```python
from build123d import *

# Parameters (mm, degrees)
SKETCH1_W                                    = 40
SKETCH1_H                                    = 430
BOSS_EXTRUDE1_DEPTH                          = 7.5
SKETCH2_R                                    = 6.5
CUT_EXTRUDE1_DEPTH                           = 3
HEX_SOCKET_CAP_SCREW_HOLE_TYPE_1_D           = 6.6
HEX_SOCKET_CAP_SCREW_HOLE_TYPE_1_CBORE_D     = 11
HEX_SOCKET_CAP_SCREW_HOLE_TYPE_1_CBORE_DEPTH = 6.8
M5_TAPPED_HOLE1_D                            = 4.2
M5_TAPPED_HOLE1_DEPTH                        = 15
M5_TAPPED_HOLE1_TIP                          = 1.2618073
CHAMFER1_SIZE                                = 2
HEX_SOCKET_CAP_SCREW_HOLE_TYPE_2_D           = 6.6
HEX_SOCKET_CAP_SCREW_HOLE_TYPE_2_CBORE_D     = 11
HEX_SOCKET_CAP_SCREW_HOLE_TYPE_2_CBORE_DEPTH = 6.8
M6_TAPPED_HOLE1_D                            = 5
M6_TAPPED_HOLE1_DEPTH                        = 13
M6_TAPPED_HOLE1_TIP                          = 1.502151548
M6_TAPPED_HOLE2_D                            = 5
M6_TAPPED_HOLE2_DEPTH                        = 13
M6_TAPPED_HOLE2_TIP                          = 1.502151548
F_6_0_6_DIAMETER_HOLE1_D                     = 6
F_6_0_6_DIAMETER_HOLE1_DEPTH                 = 17
F_6_0_6_DIAMETER_HOLE1_TIP                   = 1.802581857


with BuildPart() as part:
    # Sketch1 → Boss-Extrude1 (new, symmetric)
    with BuildSketch(Plane(origin=(0, 0, 0), x_dir=(1, 0, 0), z_dir=(0, 1, 0))):
        Rectangle(SKETCH1_W, SKETCH1_H)
    extrude(amount=BOSS_EXTRUDE1_DEPTH, both=True)

    # Sketch2 → Cut-Extrude1 (cut)
    with BuildSketch(Plane(origin=(0, 7.5, 0), x_dir=(1, 0, 0), z_dir=(0, 1, 0))):
        with Locations(Location((0, 195, 0), (0, 0, 270))):
            Circle(SKETCH2_R)
        with Locations(Location((0, -195, 0), (0, 0, 90))):
            Circle(SKETCH2_R)
    extrude(amount=-CUT_EXTRUDE1_DEPTH, mode=Mode.SUBTRACT)

    # Hex socket cap screw hole type 1 (through all)
    with Locations(Plane(origin=(0, -7.5, 0), x_dir=(-1, 0, 0), z_dir=(0, -1, 0))):
        with Locations((0, -195), (0, 195)):
            CounterBoreHole(HEX_SOCKET_CAP_SCREW_HOLE_TYPE_1_D / 2, HEX_SOCKET_CAP_SCREW_HOLE_TYPE_1_CBORE_D / 2, HEX_SOCKET_CAP_SCREW_HOLE_TYPE_1_CBORE_DEPTH)

    # M5 Tapped Hole1
    with Locations(Plane.ZY.offset(20)):
        with Locations((-195, 0), (195, 0), (-65, 0), (65, 0)):
            Hole(M5_TAPPED_HOLE1_D / 2, depth=M5_TAPPED_HOLE1_DEPTH)
            with Locations((0, 0, -(M5_TAPPED_HOLE1_DEPTH + M5_TAPPED_HOLE1_TIP / 2))):  # 118° drill point
                Cone(0, M5_TAPPED_HOLE1_D / 2, M5_TAPPED_HOLE1_TIP, mode=Mode.SUBTRACT)

    # Chamfer1
    chamfer1_edges = [part.edges().sort_by_distance(p)[0] for p in [
        (-20, 0, -215),
        (20, 0, -215),
        (20, 0, 215),
        (-20, 0, 215),
    ]]
    chamfer(chamfer1_edges, length=CHAMFER1_SIZE)

    # Hex socket cap screw hole type 2 (through all)
    with Locations(Plane(origin=(0, 7.5, 0), x_dir=(1, 0, 0), z_dir=(0, 1, 0))):
        with Locations((0, 175), (0, -175), (0, 0)):
            CounterBoreHole(HEX_SOCKET_CAP_SCREW_HOLE_TYPE_2_D / 2, HEX_SOCKET_CAP_SCREW_HOLE_TYPE_2_CBORE_D / 2, HEX_SOCKET_CAP_SCREW_HOLE_TYPE_2_CBORE_DEPTH)

    # M6 Tapped Hole1
    with Locations(Plane.XY.offset(215)):
        with Locations((0, 0)):
            Hole(M6_TAPPED_HOLE1_D / 2, depth=M6_TAPPED_HOLE1_DEPTH)
            with Locations((0, 0, -(M6_TAPPED_HOLE1_DEPTH + M6_TAPPED_HOLE1_TIP / 2))):  # 118° drill point
                Cone(0, M6_TAPPED_HOLE1_D / 2, M6_TAPPED_HOLE1_TIP, mode=Mode.SUBTRACT)

    # M6 Tapped Hole2
    with Locations(Plane(origin=(0, 0, -215), x_dir=(-1, 0, 0), z_dir=(0, 0, -1))):
        with Locations((0, 0)):
            Hole(M6_TAPPED_HOLE2_D / 2, depth=M6_TAPPED_HOLE2_DEPTH)
            with Locations((0, 0, -(M6_TAPPED_HOLE2_DEPTH + M6_TAPPED_HOLE2_TIP / 2))):  # 118° drill point
                Cone(0, M6_TAPPED_HOLE2_D / 2, M6_TAPPED_HOLE2_TIP, mode=Mode.SUBTRACT)

    # Ø6.0 (6) Diameter Hole1
    with Locations(Plane(origin=(0, -7.5, 0), x_dir=(-1, 0, 0), z_dir=(0, -1, 0))):
        with Locations((0, 100), (0, -100)):
            Hole(F_6_0_6_DIAMETER_HOLE1_D / 2, depth=F_6_0_6_DIAMETER_HOLE1_DEPTH)
            with Locations((0, 0, -(F_6_0_6_DIAMETER_HOLE1_DEPTH + F_6_0_6_DIAMETER_HOLE1_TIP / 2))):  # 118° drill point
                Cone(0, F_6_0_6_DIAMETER_HOLE1_D / 2, F_6_0_6_DIAMETER_HOLE1_TIP, mode=Mode.SUBTRACT)


solid = part.part
```
Geometry check sheet. Reference: the model listing, model coordinates, mm. A direction names the side the tool comes from. Coordinates: 2 decimals unless noted, no trailing zeros.
Q1. Tool access check on faces 4 (the face through (-0.72, 1.94, -191.78)), 5 (the face through (-1.19, 4.15, -169.63)), 6 (the face through (4.4, -4.1, -191.7)). Record the directions out of +Z, -Z, +X, -X, +Y, -Y that give a thin tool (end or side, any length) a straight path to the whole face; none if there is none.
Reply:
face 4: +Y, -Y
face 5: +Y
face 6: -Y
Q2. Depth check by flat-ended pin: pin 1 Ø14.5 at (x, z) = (0, 0) entering from -Y; pin 2 Ø2.5 at (y, z) = (0, -195) entering from -X; pin 3 Ø10.5 at (x, z) = (0, 195) entering from -Y; pin 4 Ø4.5 at (x, y) = (0, 0) entering from -Z. Enter the tip coordinate at first touch or a pass-through.
Reply:
pin 1: stops at y = -7.5
pin 2: stops at x = -4.49
pin 3: stops at y = -0.7
pin 4: stops at z = -201.85
Q3. Thickness scan on probe 1 along X at (y, z) = (5.1, 195); probe 2 along Y at (x, z) = (-16, -65); probe 3 along X at (y, z) = (0, 207.5). Record the ranges inside material, lowest first.
Reply:
probe 1: x = -20 to -6.5, 6.5 to 20
probe 2: y = -7.5 to -2.1, 2.1 to 7.5
probe 3: x = -20 to -2.5, 2.5 to 20
Q4. Draft check along Z on faces 1 (the face through (2.43, -3.46, -2.23)), 2 (the face through (0, 3, 215)), 3 (the face through (-5, -7.5, -3)). Enter one of: released by +Z, released by -Z, zero draft, split by the parting line, or undercut.
Reply:
face 1: undercut
face 2: released by +Z
face 3: zero draft
